CAD build for the part. Positions are in the model's coordinates, mm. A direction names the side the tool comes from. Give positions to 0.01 mm unless a question says otherwise; leave off trailing zeros. Order: outer loops, then holes, each group sorted by start corner. A loop starts at its lowest first (then second) coordinate and runs counter-clockwise, first axis right, second up. Notation, with made-up numbers: M -7,76 L 38,76 A12 cw 38,86 Z; hole C 55.25,-5.5 d2. An arc over 180 degrees is marked long. Put each result on its own line as item: value. Start each with the question number.
1) Drill centre lines: line 1 (Z direction, x = 61, y = 17); line 2 (X direction, y = 33, z = 136); line 3 (Y direction, x = 59, z = 142). Where is each one in solid material? Low to high. Write a range as [from, to].
2) Two-plate mould, pull along X, no slides. Class faces 1 (the face through (23.832, 13.748, 127.357)), 2 (the face through (45, 17, 105.373)), 3 (the face through (0, 30, 9)): released by +X, released by -X, zero draft, split by the parting line, or undercut.
3) Pin check, flat tips, straight feed: pin 1 (3 mm diameter, centred on y = 19, z = 127, fed in from +X); pin 2 (1 mm diameter, centred on y = 24.5, z = 70.5, fed in from +X); pin 3 (10.5 mm diameter, centred on x = 34.5, z = 110.5, fed in from -Y); pin 4 (18 mm diameter, centred on x = 72, y = 60, fed in from +Z). Stop position of each tip, or through.
4) Cut at B-B (z = 160.5). Write the cut outline in (x, y), and give its area (3 significant figures).
5) Cut at A-A (y = 17). Write the cut outline in (x, z), and give its area (3 significant figures).
6) Cut at D-D (z = 142). Write the cut outline in (x, y).
7) Cut at C-C (x = 46). Write the cut outline in (y, z), and give its area (3 significant figures).
8) Tool access for faces 4 (the face through (45, 40, 38)), 5 (the face through (78, 23, 156)), 6 (the face through (45, 0, 104)): list every direction of +Z, -Z, +X, -X, +Y, -Y with a clear straight run to the whole face (end or side of a thin tool).
```python
from build123d import *

# Parameters (mm, degrees)
MOUNTING_PLATE_SKETCH_R       = 10
MOUNTING_PLATE_DEPTH          = 18
ARM_START                     = -20
ARM_SKETCH_40X40_W            = 40
ARM_SKETCH_40X40_H            = 40
ARM_BOSS_DEPTH                = 54
ARM_EXTENSION_SKETCH_W        = 62
ARM_EXTENSION_SKETCH_H        = 34
ARM_EXTENSION_DEPTH           = 54
ARM_RECESS_SKETCH_W           = 60
ARM_RECESS_SKETCH_H           = 22
ARM_RECESS_CUT_DEPTH          = 54
STEP_PAD_DEPTH                = 6
STEP_PAD_DEPTH_BACK           = 60
STEP_PAD_SKETCH_R             = 30
STEP_PAD_SKETCH_R_2           = 15
CLEVIS_PROFILE_CUT_DEPTH      = 211.82694325
CLEVIS_PROFILE_CUT_DEPTH_BACK = 211.82694325
CLEVIS_PROFILE_SKETCH_W       = 18
CLEVIS_PROFILE_SKETCH_H       = 63.461103314
CLEVIS_SLOT_CUT_DEPTH         = 201.641471286
CLEVIS_SLOT_CUT_DEPTH_BACK    = 201.641471286
CLEVIS_SLOT_SKETCH_W          = 18
CLEVIS_SLOT_SKETCH_H          = 11.909045211


with BuildPart() as part:
    # Mounting Plate Sketch → Mounting Plate (new body)
    with BuildSketch(Plane.XY):
        with BuildLine():
            Line((0, 0), (92, 0))
            Line((92, 0), (92, 60))
            ThreePointArc((92, 60), (86.142135624, 74.142135624), (72, 80))
            Line((72, 80), (20, 80))
            ThreePointArc((20, 80), (5.857864376, 74.142135624), (0, 60))
            Line((0, 60), (0, 0))
        make_face()
        with Locations((20, 60)):
            Circle(MOUNTING_PLATE_SKETCH_R, mode=Mode.SUBTRACT)
        with Locations((72, 60)):
            Circle(MOUNTING_PLATE_SKETCH_R, mode=Mode.SUBTRACT)
    extrude(amount=MOUNTING_PLATE_DEPTH)

    # Arm Sketch 40x40 → Arm Boss (add)
    with BuildSketch(Plane(origin=(92, 0, 0), x_dir=(0, 0, -1), z_dir=(1, 0, 0)).offset(ARM_START)):
        with Locations((-38, 20)):
            Rectangle(ARM_SKETCH_40X40_W, ARM_SKETCH_40X40_H)
    extrude(amount=-ARM_BOSS_DEPTH)

    # Arm Extension Sketch → Arm Extension (add)
    with BuildSketch(Plane(origin=(72, 0, 0), x_dir=(0, 0, -1), z_dir=(1, 0, 0))):
        with Locations((-89, 17)):
            Rectangle(ARM_EXTENSION_SKETCH_W, ARM_EXTENSION_SKETCH_H)
    extrude(amount=-ARM_EXTENSION_DEPTH)

    # Arm Recess Sketch → Arm Recess Cut (cut)
    with BuildSketch(Plane(origin=(72, 0, 0), x_dir=(0, 0, -1), z_dir=(1, 0, 0))):
        with Locations((-66, 11)):
            Rectangle(ARM_RECESS_SKETCH_W, ARM_RECESS_SKETCH_H)
    extrude(amount=-ARM_RECESS_CUT_DEPTH, mode=Mode.SUBTRACT)

    # Step Pad Sketch → Step Pad (add, two sides: drawn at the far end of the back side and taken through both)
    with BuildSketch(Plane(origin=(72, 0, 0), x_dir=(0, 0, -1), z_dir=(1, 0, 0)).offset(-STEP_PAD_DEPTH_BACK)):
        with Locations(Location((-142, 17, 0), (0, 0, 90))):
            Circle(STEP_PAD_SKETCH_R)
        with Locations(Location((-142, 17, 0), (0, 0, 90))):
            Circle(STEP_PAD_SKETCH_R_2, mode=Mode.SUBTRACT)
    extrude(amount=STEP_PAD_DEPTH + STEP_PAD_DEPTH_BACK)

    # Clevis Profile Sketch → Clevis Profile Cut (cut, two sides: drawn at the far end of the back side and taken through both)
    with BuildSketch(Plane(origin=(0, 0, 0), x_dir=(1, 0, 0), z_dir=(0, 1, 0)).offset(-CLEVIS_PROFILE_CUT_DEPTH_BACK)):
        with Locations((45, -149.012137468)):
            Rectangle(CLEVIS_PROFILE_SKETCH_W, CLEVIS_PROFILE_SKETCH_H)
    extrude(amount=CLEVIS_PROFILE_CUT_DEPTH + CLEVIS_PROFILE_CUT_DEPTH_BACK, mode=Mode.SUBTRACT)

    # Clevis Slot Sketch → Clevis Slot Cut (cut, two sides: drawn at the far end of the back side and taken through both)
    with BuildSketch(Plane(origin=(0, 34, 0), x_dir=(1, 0, 0), z_dir=(0, 1, 0)).offset(-CLEVIS_SLOT_CUT_DEPTH_BACK)):
        with Locations((45, -111.327063206)):
            Rectangle(CLEVIS_SLOT_SKETCH_W, CLEVIS_SLOT_SKETCH_H)
    extrude(amount=CLEVIS_SLOT_CUT_DEPTH + CLEVIS_SLOT_CUT_DEPTH_BACK, mode=Mode.SUBTRACT)


solid = part.part
```
Solution:
1. line 1: [0, 36], [96, 127], [157, 172]
1. line 2: [12, 36], [54, 78]
1. line 3: [-13, 2], [32, 47]
2. face 1: zero draft
2. face 2: undercut
2. face 3: released by -X
3. pin 1: x = 78
3. pin 2: x = 72
3. pin 3: y = 0
3. pin 4: through
4. outline: M 12,-6.62 L 36,-6.62 L 36,40.62 L 12,40.62 Z; M 54,-6.62 L 78,-6.62 L 78,40.62 L 54,40.62 Z
4. area: 2,270 mm²
5. outline: M 0,0 L 92,0 L 92,18 L 72,18 L 72,36 L 18,36 L 18,18 L 0,18 Z; M 12,112 L 18,112 L 18,96 L 72,96 L 72,112 L 78,112 L 78,127 L 54,127 L 54,105.37 L 36,105.37 L 36,127 L 12,127 Z; M 12,157 L 36,157 L 36,172 L 12,172 Z; M 54,157 L 78,157 L 78,172 L 54,172 Z
5. area: 4,810 mm²
6. outline: M 12,-13 L 36,-13 L 36,2 L 12,2 Z; M 12,32 L 36,32 L 36,47 L 12,47 Z; M 54,-13 L 78,-13 L 78,2 L 54,2 Z; M 54,32 L 78,32 L 78,47 L 54,47 Z
7. outline: M 0,0 L 80,0 L 80,18 L 40,18 L 40,58 L 34,58 L 34,105.37 L 0,105.37 L 0,96 L 22,96 L 22,36 L 0,36 Z
7. area: 3,330 mm²
8. face 4: +X, -X, +Y
8. face 5: +Z, +X, +Y, -Y
8. face 6: -Z, +X, -X, -Y
